from build123d import *

# Parameters (mm, degrees)
BOSS_EXTRUDE1_DEPTH = 9
BOSS_EXTRUDE2_START = 15
SKETCH5_R           = 10
BOSS_EXTRUDE2_DEPTH = 15
CHAMFER1_SIZE       = 1


with BuildPart() as part:
    # Sketch1 → Revolve1 (revolve)
    with BuildSketch(Plane.XY, mode=Mode.PRIVATE) as revolve1_sk:
        Polygon((35, 0), (60, 0), (60, 9.5), (59.5, 10), (60, 10.5), (60, 20), (42, 20), (21, 31), (10, 31), (10, 181), (0, 181), (0, 15), (14, 15), align=None)
    revolve(revolve1_sk.sketch.rotate(Axis((0, 181, 0), (0, -1, 0)), 180), axis=Axis((0, 181, 0), (0, -1, 0)))

    # Sketch2 → Boss-Extrude1 (add)
    with BuildSketch(Plane(origin=(0, 31, 0), x_dir=(1, 0, 0), z_dir=(0, 1, 0))):
        Polygon((12, 6.92820323), (0, 13.856406461), (-12, 6.92820323), (-12, -6.92820323), (0, -13.856406461), (12, -6.92820323), align=None)
    extrude(amount=BOSS_EXTRUDE1_DEPTH)

    # Sketch3 → Cut-Revolve1 (revolve, cut)
    with BuildSketch(Plane(origin=(0, 0, 0), x_dir=(0, 0, -1), z_dir=(1, 0, 0))):
        Polygon((12.356406461, 31), (13.856406461, 31.866025404), (13.856406461, 31), align=None)
        Polygon((13.856406461, 39.422649731), (12.856406461, 40), (13.856406461, 40), align=None)
    revolve(axis=Axis((0, 181, 0), (0, 1, 0)), mode=Mode.SUBTRACT)

    # Sketch5 → Boss-Extrude2 (add)
    with BuildSketch(Plane(origin=(0, 41, 0), x_dir=(-1, 0, 0), z_dir=(0, 1, 0)).offset(BOSS_EXTRUDE2_START)):
        Polygon((0, 19.225763964), (-16.65, 9.612881982), (-16.65, -9.612881982), (0, -19.225763964), (16.65, -9.612881982), (16.65, 9.612881982), align=None)
        with Locations(Location((0, 0, 0), (0, 0, 90))):
            Circle(SKETCH5_R, mode=Mode.SUBTRACT)
    extrude(amount=-BOSS_EXTRUDE2_DEPTH)

    # Sketch7 → Cut-Revolve3 (revolve, cut)
    with BuildSketch(Plane(origin=(0, 0, 0), x_dir=(0, 0, -1), z_dir=(1, 0, 0)), mode=Mode.PRIVATE) as cut_revolve3_sk:
        Polygon((16.525763964, 56), (19.225763964, 53.3), (19.225763964, 56), align=None)
        Polygon((16.525763964, 41), (19.225763964, 43.7), (19.225763964, 41), align=None)
    revolve(cut_revolve3_sk.sketch.rotate(Axis((0, 181, 0), (0, 1, 0)), 180), axis=Axis((0, 181, 0), (0, 1, 0)), mode=Mode.SUBTRACT)

    # Chamfer1
    chamfer1_edges = [part.edges().sort_by_distance(p)[0] for p in [
        (10, 181, 0),
    ]]
    chamfer(chamfer1_edges, length=CHAMFER1_SIZE)


solid = part.part
Work out the finished part from the listing and answer in its coordinate system (mm). A direction names the side the tool comes from. Give positions to 0.01 mm unless a question says otherwise; leave off trailing zeros. Order: outer loops, then holes, each group sorted by start corner. A loop starts at its lowest first (then second) coordinate and runs counter-clockwise, first axis right, second up. Notation, with made-up numbers: (89.5, 69) - (95.5, 69) arc R18 ccw to (95.5, 91) - close; hole circle Ø3 at (43.5, -3.75). An arc over 180 degrees is marked (long way). Answer as CSV lines item,"result". Start each with the question number.
Q1. The mould has two halves that part along Y. Classify faces 1 (the face through (0.73, 55.83, -16.68)), 2 (the face through (16.65, 49, 0)), 3 (the face through (-9, 31, 9)): +Y half, -Y half, draft (parallel to the pull), parting line (faces both ways), or undercut.
Q2. The part is cut by section A-A (y = 147). Write down the section's boundary in (x, z).
Q3. For faces 4 (the face through (-8.442, 48.603, 14.352)), 5 (the face through (-16.65, 49, 0)), 6 (the face through (0.73, 41.17, -16.68)), determine the directions among +Z, -Z, +X, -X, +Y, -Y from which every point of the face is accessible in a straight line to the end or side of a thin tool.
Q4. Given pin 1 Ø4.5 at (y, z) = (35, 1) entering from -X; pin 2 Ø4 at (x, z) = (-27.5, 1) entering from -Y; pin 3 Ø2 at (x, z) = (-33.5, -24.5) entering from +Y, each flat-ended and moving along its own axis, determine where each tip first touches the part or whether it passes through.
Q5. Find the intervals of material crossed by L1, parallel to Y at x = 41.5, z = 25; L2, parallel to X at y = 52.5, z = -9.5; L3, parallel to Z at x = 9, y = 28.5, in increasing order. Write a range as [from, to].
Check result:
1,face 1,"+Y half"
1,face 2,"draft"
1,face 3,"undercut"
2,outline,"circle Ø20 at (0, 0)"
3,face 4,"+Z, -X, +Y"
3,face 5,"+Z, -Z, -X, +Y"
3,face 6,"none"
4,pin 1,"stops at x = -12"
4,pin 2,"stops at y = 3.92"
4,pin 3,"stops at y = 20.78"
5,L1,"y = [0, 20]"
5,L2,"x = [-16.65, 16.65]"
5,L3,"z = [-24.15, 24.15]"
